Can you work these out from the model? Positions are in its coordinate system, mm. A direction names the side the tool comes from. Give positions to 0.01 mm unless a question says otherwise; leave off trailing zeros. Order: outer loops, then holes, each group sorted by start corner. A loop starts at its lowest first (then second) coordinate and runs counter-clockwise, first axis right, second up. Notation, with made-up numbers: M 82,-6 L 141,-6 A15 cw 141,6 Z; hole C -25,81 d9. An arc over 180 degrees is marked long. Write each question's results on one line, items separated by ' | '.
from build123d import *

# Parameters (mm, degrees)
TUBE_PROFILE_50X50X5_SKETCH_W   = 50
TUBE_PROFILE_50X50X5_SKETCH_H   = 50
TUBE_PROFILE_50X50X5_SKETCH_W_2 = 40
TUBE_PROFILE_50X50X5_SKETCH_H_2 = 40
SQUARE_TUBE_BODY_L90_DEPTH      = 90
KEYHOLE_NOTCH_SKETCH_W          = 8
KEYHOLE_NOTCH_SKETCH_H          = 10
KEYHOLE_NOTCHES_DEPTH           = 5
OBROUND_BOSS_DEPTH              = 7
OBROUND_START                   = -7
OBROUND_SLOT_CUT_DEPTH          = 7
SIDE_BOSS_AND_HOLES_SKETCH_R    = 12.5
SIDE_BOSS_AND_HOLES_SKETCH_R_2  = 9.5
SIDE_BOSS_25_DEPTH              = 12
SKETCH7_3_R                     = 4
SKETCH7_3_R_2                   = 9.5
SIDE_BORE_AND_HOLES_DEPTH       = 108.814655776


with BuildPart() as part:
    # Tube Profile 50x50x5 Sketch → Square Tube Body L90 (new body)
    with BuildSketch(Plane.XY):
        Rectangle(TUBE_PROFILE_50X50X5_SKETCH_W, TUBE_PROFILE_50X50X5_SKETCH_H)
        Rectangle(TUBE_PROFILE_50X50X5_SKETCH_W_2, TUBE_PROFILE_50X50X5_SKETCH_H_2, mode=Mode.SUBTRACT)
    extrude(amount=SQUARE_TUBE_BODY_L90_DEPTH)

    # Keyhole Notch Sketch → Keyhole Notches (cut)
    with BuildSketch(Plane(origin=(0, 25, 0), x_dir=(1, 0, 0), z_dir=(0, 1, 0))):
        with BuildLine():
            Line((14, -90), (14, -80))
            ThreePointArc((14, -80), (10, -76), (6, -80))
            Line((6, -80), (6, -90))
            Line((6, -90), (14, -90))
        make_face()
        with Locations((-14, -5)):
            Rectangle(KEYHOLE_NOTCH_SKETCH_W, KEYHOLE_NOTCH_SKETCH_H)
    extrude(amount=-KEYHOLE_NOTCHES_DEPTH, mode=Mode.SUBTRACT)

    # Obround Boss Sketch → Obround Boss (add)
    with BuildSketch(Plane(origin=(0, 25, 0), x_dir=(1, 0, 0), z_dir=(0, 1, 0))):
        with BuildLine():
            Line((15, -35), (15, -55))
            ThreePointArc((15, -55), (0, -70), (-15, -55))
            Line((-15, -55), (-15, -35))
            ThreePointArc((-15, -35), (0, -20), (15, -35))
        make_face()
        with BuildLine():
            Line((10, -35), (10, -55))
            ThreePointArc((10, -55), (0, -65), (-10, -55))
            Line((-10, -55), (-10, -35))
            ThreePointArc((-10, -35), (0, -25), (10, -35))
        make_face(mode=Mode.SUBTRACT)
    extrude(amount=OBROUND_BOSS_DEPTH)

    # Sketch6_2 → Obround Slot Cut (cut)
    with BuildSketch(Plane(origin=(0, 25, 0), x_dir=(1, 0, 0), z_dir=(0, 1, 0)).offset(OBROUND_START)):
        with BuildLine():
            Line((10, -35), (10, -55))
            ThreePointArc((10, -55), (0, -65), (-10, -55))
            Line((-10, -55), (-10, -35))
            ThreePointArc((-10, -35), (0, -25), (10, -35))
        make_face()
    extrude(amount=OBROUND_SLOT_CUT_DEPTH, mode=Mode.SUBTRACT)

    # Side Boss and Holes Sketch → Side Boss _25 (add)
    with BuildSketch(Plane(origin=(25, 0, 0), x_dir=(0, 0, -1), z_dir=(1, 0, 0))):
        with Locations(Location((-45, 0, 0), (0, 0, 270))):
            Circle(SIDE_BOSS_AND_HOLES_SKETCH_R)
        with Locations(Location((-45, 0, 0), (0, 0, 90))):
            Circle(SIDE_BOSS_AND_HOLES_SKETCH_R_2, mode=Mode.SUBTRACT)
    side_boss_25 = extrude(amount=SIDE_BOSS_25_DEPTH)

    # Sketch7_3 → Side Bore and Holes (cut, through all)
    with BuildSketch(Plane(origin=(25, 0, 0), x_dir=(0, 0, -1), z_dir=(1, 0, 0))):
        with Locations(Location((-80, 0, 0), (0, 0, 90))):
            Circle(SKETCH7_3_R)
        with Locations(Location((-10, 0, 0), (0, 0, 90))):
            Circle(SKETCH7_3_R)
        with Locations(Location((-45, 0, 0), (0, 0, 270))):
            Circle(SKETCH7_3_R_2)
    extrude(amount=-SIDE_BORE_AND_HOLES_DEPTH, mode=Mode.SUBTRACT)

    # Side Boss Mirror: Side Boss _25 across plane
    add(side_boss_25.mirror(Plane(origin=(0, 0, 0), x_dir=(0, 0, 1), z_dir=(1, 0, 0))))


solid = part.part
(1) Imagine slicing it at B-B, the plane y = 17. Write out the boundary of the cut face in (x, z).
Data:
outline: M -25,0 L -20,0 L -20,90 L -25,90 Z; M 20,0 L 25,0 L 25,90 L 20,90 Z
(2) For faces 4 (the face through (30.916, 2.71, 57.203)), 5 (the face through (16, 25, 44)), 6 (the face through (-14, 20, 44)), which set-ups out of +Z, -Z, +X, -X, +Y, -Y let a thin tool reach every point of the face, with its end or its side?
Data:
face 4: +X | face 5: +Y | face 6: +Z, -Z
(3) I need wall thicknesses on L1, parallel to Z at x = 22.1, y = 0; L2, parallel to X at y = -14, z = 28; L3, parallel to Y at x = -29, z = 45. Which ranges of each line are inside material? Lowest first, please. Write a range as from..to.
Data:
L1: z = 0..6, 14..35.5, 54.5..76, 84..90 | L2: x = -25..-20, 20..25 | L3: y = -12.5..-9.5, 9.5..12.5
(4) Will these pins go through, and if not, where does the flat tip stop? P1, Ø10, axis at y = -14.5, z = 30.5, coming from the +X side; P2, Ø9, axis at y = 0, z = 10, coming from the -X side; P3, Ø12, axis at y = -1.5, z = 48.5, coming from the -X side; P4, Ø11.5, axis at y = 0, z = 45, coming from the +X side.
Data:
P1: stops at x = 25 | P2: stops at x = -25 | P3: stops at x = -37 | P4: passes through
(5) Imagine slicing it at C-C, the plane y = 27.5. Write out the boundary of the cut face in (x, z).
Data:
outline: M -15,35 A15 ccw 15,35 L 15,55 A15 ccw -15,55 Z; hole M -10,35 A10 ccw 10,35 L 10,55 A10 ccw -10,55 Z
(6) Imagine slicing it at A-A, the plane z = 45. Count the separate pieces of the cut face and the enclosed holes in it, plus the area to 3 significant figures.
Data:
separate pieces: 3 | enclosed holes: 0 | area: 824 mm2
(7) We'd pull the mould along X, two halves only. Please class faces 1 (the face through (-22.465, -0.521, 13.966)), 2 (the face through (0, 28, 70)), 3 (the face through (0, 26, 25)): +X half, -X half, draft (parallel to the pull), parting line (faces both ways), or undercut.
Data:
face 1: draft | face 2: parting line | face 3: undercut
